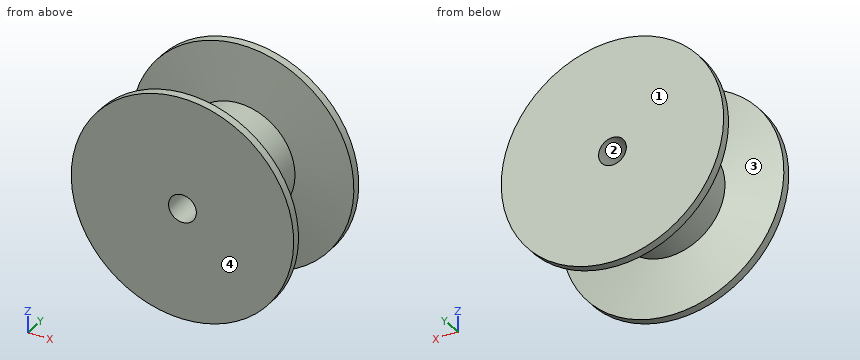
from build123d import *


with BuildPart() as part:
    # 草图1 → 旋转1 (revolve)
    with BuildSketch(Plane(origin=(0, 0, 0), x_dir=(0, 0, -1), z_dir=(1, 0, 0))):
        Polygon((5, 0), (40, 0), (40, 3), (20, 5), (20, 35), (40, 37), (40, 40), (5, 40), align=None)
    revolve(axis=Axis((0, 0, 0), (0, 1, 0)))


solid = part.part
Verification items for the finished model (mm, model axes). Face numbers are marked on the shaded views. Coordinates: 2 decimals unless noted, no trailing zeros. Loops run counter-clockwise (first coordinate to the right, second up) from the corner with the lowest first, then second, coordinate; pieces in that order, holes last. Notation, with made-up numbers: M -28,7.5 L -7,7.5 A14 ccw -7,12.5 Z; hole C 68,20.25 d6. An arc over 180 degrees is marked long. One line per item, written item: value.
1. Mould release check, pull along Y, two halves, no side actions. Record for the marked faces 1, 2, 3 and 4: pulls with the +Y half, pulls with the -Y half, needs draft (parallel to the pull), parting line crosses it, or undercut.
Answers follow:
face 1: pulls with the +Y half
face 2: needs draft
face 3: undercut
face 4: pulls with the -Y half
2. Section check C-C on y = 31. Record the cut outline in (x, z).
Answers follow:
outline: C 0,0 d40; hole C 0,0 d10
3. Section check B-B on x = 0. Record the cut outline in (y, z).
Answers follow:
outline: M 0,-40 L 3,-40 L 5,-20 L 35,-20 L 37,-40 L 40,-40 L 40,-5 L 0,-5 Z; M 0,5 L 40,5 L 40,40 L 37,40 L 35,20 L 5,20 L 3,40 L 0,40 Z
4. Material ranges on line 1 along Z through (x, y) = (0, 30); line 2 along Y through (x, z) = (1, -26), recorded low to high. Write a range as from..to.
Answers follow:
line 1: -20..-5, 5..20
line 2: 0..4.4, 35.6..40
5. Section check A-A on z = 0. Record the cut outline in (x, y).
Answers follow:
outline: M -40,0 L -5,0 L -5,40 L -40,40 L -40,37 L -20,35 L -20,5 L -40,3 Z; M 5,0 L 40,0 L 40,3 L 20,5 L 20,35 L 40,37 L 40,40 L 5,40 Z
6. Gauge pin test, flat ends, axial feed: P1, Ø12, axis at x = -7, y = 17.5, coming from the +Z side (3 decimals); P2, Ø10, axis at x = 17, y = 33, coming from the +Z side; P3, Ø6, axis at x = 0, z = 0, coming from the -Y side; P4, Ø10, axis at y = 18.5, z = 6, coming from the +X side (3 decimals). Record the tip position at first contact, or that the pin passes through.
Answers follow:
P1: z = 19.975
P2: z = 37.47
P3: through
P4: x = 19.975
